Work out the finished part from the listing and answer in its coordinate system (mm). A direction names the side the tool comes from. Coordinates: 2 decimals unless noted, no trailing zeros. Order: outer loops, then holes, each group sorted by start corner. A loop starts at its lowest first (then second) coordinate and runs counter-clockwise, first axis right, second up. Notation, with made-up numbers: (-5, 43.5) -> (28, 43.5) arc R9 ccw to (28, 54.5) -> close; hole circle Ø11 at (41, -6). An arc over 180 degrees is marked (long way). Use one line per item in the form item = value.
from build123d import *

# Parameters (mm, degrees)
BASE_PLATE_SKETCH_W     = 100
BASE_PLATE_SKETCH_H     = 100
BASE_PLATE_DEPTH        = 20
FLANGE_DISC_SKETCH_R    = 50
FLANGE_DISC_DEPTH       = 5
FLANGE_HOLES_SKETCH_R   = 4
FLANGE_HOLES_4X_8_DEPTH = 5
HUB_DISC_SKETCH_R       = 35
HUB_DISC_DEPTH          = 5
ARC_SLOTS_3X_DEPTH      = 5
CENTRE_BORE_SKETCH_R    = 15
CENTRE_BORE_DEPTH       = 10


with BuildPart() as part:
    # Base Plate Sketch → Base Plate (new body)
    with BuildSketch(Plane(origin=(0, 0, 0), x_dir=(1, 0, 0), z_dir=(0, 1, 0))):
        Rectangle(BASE_PLATE_SKETCH_W, BASE_PLATE_SKETCH_H)
    extrude(amount=BASE_PLATE_DEPTH)

    # Flange Disc Sketch → Flange Disc (add)
    with BuildSketch(Plane(origin=(0, 20, 0), x_dir=(1, 0, 0), z_dir=(0, 1, 0))):
        with Locations(Location((0, 0, 0), (0, 0, 270))):
            Circle(FLANGE_DISC_SKETCH_R)
    extrude(amount=FLANGE_DISC_DEPTH)

    # Flange Holes Sketch → Flange Holes 4xØ8 (cut)
    with BuildSketch(Plane(origin=(0, 25, 0), x_dir=(1, 0, 0), z_dir=(0, 1, 0))):
        with Locations(Location((0, 41.5, 0), (0, 0, 270))):
            Circle(FLANGE_HOLES_SKETCH_R)
        with Locations(Location((41.5, 0, 0), (0, 0, 270))):
            Circle(FLANGE_HOLES_SKETCH_R)
        with Locations(Location((0, -41.5, 0), (0, 0, 270))):
            Circle(FLANGE_HOLES_SKETCH_R)
        with Locations(Location((-41.5, 0, 0), (0, 0, 270))):
            Circle(FLANGE_HOLES_SKETCH_R)
    extrude(amount=-FLANGE_HOLES_4X_8_DEPTH, mode=Mode.SUBTRACT)

    # Hub Disc Sketch → Hub Disc (add)
    with BuildSketch(Plane(origin=(0, 25, 0), x_dir=(1, 0, 0), z_dir=(0, 1, 0))):
        with Locations(Location((0, 0, 0), (0, 0, 270))):
            Circle(HUB_DISC_SKETCH_R)
    extrude(amount=HUB_DISC_DEPTH)

    # Arc Slots Sketch → Arc Slots 3x (cut)
    with BuildSketch(Plane(origin=(0, 30, 0), x_dir=(1, 0, 0), z_dir=(0, 1, 0))):
        with BuildLine():
            ThreePointArc((-27.405227761, -12.2046504), (-16.338, -25.160877489), (0, -30))
            ThreePointArc((0, -30), (5, -25), (0, -20))
            ThreePointArc((0, -20), (-10.892, -16.773918326), (-18.27015184, -8.1364336))
            ThreePointArc((-18.27015184, -8.1364336), (-24.871798201, -5.60300404), (-27.405227761, -12.2046504))
        make_face()
        with BuildLine():
            ThreePointArc((16.773411359, 10.8927807), (18.243569024, 17.809328715), (25.160117038, 16.33917105))
            ThreePointArc((25.160117038, 16.33917105), (30, 0), (25.160117038, -16.33917105))
            ThreePointArc((25.160117038, -16.33917105), (18.243569024, -17.809328715), (16.773411359, -10.8927807))
            ThreePointArc((16.773411359, -10.8927807), (20, 0), (16.773411359, 10.8927807))
        make_face()
        with BuildLine():
            ThreePointArc((0, 30), (5, 25), (0, 20))
            ThreePointArc((0, 20), (-10.892, 16.773918326), (-18.27015184, 8.1364336))
            ThreePointArc((-18.27015184, 8.1364336), (-24.871798201, 5.60300404), (-27.405227761, 12.2046504))
            ThreePointArc((-27.405227761, 12.2046504), (-16.338, 25.160877489), (0, 30))
        make_face()
    extrude(amount=-ARC_SLOTS_3X_DEPTH, mode=Mode.SUBTRACT)

    # Centre Bore Sketch → Centre Bore (cut)
    with BuildSketch(Plane(origin=(0, 30, 0), x_dir=(1, 0, 0), z_dir=(0, 1, 0))):
        with Locations(Location((0, 0, 0), (0, 0, 270))):
            Circle(CENTRE_BORE_SKETCH_R)
    extrude(amount=-CENTRE_BORE_DEPTH, mode=Mode.SUBTRACT)


solid = part.part
(1) Section D-D on x = -41.5 is taken. Write down the section's boundary in (y, z), plus the area to 3 significant figures.
Data:
outline = (0, -50) -> (20, -50) -> (20, -27.89) -> (25, -27.89) -> (25, -4) -> (20, -4) -> (20, 4) -> (25, 4) -> (25, 27.89) -> (20, 27.89) -> (20, 50) -> (0, 50) -> close
area = 2,240 mm²
(2) Which of the six approach directions +Z, -Z, +X, -X, +Y, -Y give full straight-line access (tool end or side, diameter ignored) to faces 4 (the flat face through (-40, 20, -38)), 5 (the cylindrical face through (45.466, 22.535, -0.521)), 6 (the flat face through (-40, 20, 38))?
Data:
face_4 = -Z, -X, +Y
face_5 = +Y
face_6 = +Z, -X, +Y
(3) Section A-A on y = 26.25 is taken. Write down the section's boundary in (x, z).
Data:
outline = circle Ø70 at (0, 0); hole (-27.41, -12.2) arc R30 ccw to (0, -30) arc R5 ccw to (0, -20) arc R20 cw to (-18.27, -8.14) arc R5 ccw to start; hole (-27.41, 12.2) arc R5 ccw to (-18.27, 8.14) arc R20 cw to (0, 20) arc R5 ccw to (0, 30) arc R30 ccw to start; hole circle Ø30 at (0, 0); hole (16.77, -10.89) arc R5 ccw to (25.16, -16.34) arc R30 ccw to (25.16, 16.34) arc R5 ccw to (16.77, 10.89) arc R20 cw to start
(4) Section C-C on z = 41.5 is taken. Write down the section's boundary in (x, y), plus the area to 3 significant figures.
Data:
outline = (-50, 0) -> (50, 0) -> (50, 20) -> (27.89, 20) -> (27.89, 25) -> (4, 25) -> (4, 20) -> (-4, 20) -> (-4, 25) -> (-27.89, 25) -> (-27.89, 20) -> (-50, 20) -> close
area = 2,240 mm²
(5) The mould has two halves that part along Z. Classify faces 1 (the flat face through (40, 20, 40)), 2 (the flat face through (-1, 10, 50)), 3 (the cylindrical face through (0.66, 25.07, -14.985)): released by +Z, released by -Z, zero draft, split by the parting line, or undercut.
Data:
face_1 = zero draft
face_2 = released by +Z
face_3 = undercut
(6) Each of these flat-tipped pins is pushed along its axis until it touches: P1, Ø6.5, axis at x = -0.5, z = 41, coming from the +Y side; P2, Ø15, axis at x = -37, z = 36, coming from the +Y side. Where does it stop, or does it pass through?
Data:
P1 = 20
P2 = 25
(7) Straight lines are drawn through the part: line 1 along X through (y, z) = (21.75, 0); line 2 along Z through (x, y) = (-11.5, 28); line 3 along Y through (x, z) = (-4, -37.5). For each, find the intervals that lie inside material, in ascending order.
Data:
line_1 = -50 to -45.5, -37.5 to -15, 15 to 37.5, 45.5 to 50
line_2 = -33.06 to -27.71, -16.36 to -9.63, 9.63 to 16.36, 27.71 to 33.06
line_3 = 0 to 25
(8) Section B-B on x = -24 is taken. Write down the section's boundary in (y, z), plus the area to 3 significant figures.
Data:
outline = (0, -50) -> (20, -50) -> (20, -43.86) -> (25, -43.86) -> (25, -25.48) -> (30, -25.48) -> (30, -18) -> (25, -18) -> (25, -5.31) -> (30, -5.31) -> (30, 5.31) -> (25, 5.31) -> (25, 18) -> (30, 18) -> (30, 25.48) -> (25, 25.48) -> (25, 43.86) -> (20, 43.86) -> (20, 50) -> (0, 50) -> close
area = 2,570 mm²
